Build history of the part. All positions in model axes, mm. Round coordinates to 2 decimals unless told otherwise and drop trailing zeros. Write each loop counter-clockwise with the first axis right and the second up, starting at its lowest first coordinate (ties: lowest second). Pieces come first, ordered by that corner, then holes.
Item 1: Wall check: probe 1 along Z at (x, y) = (29.5, -0.25); probe 2 along Z at (x, y) = (25.5, 5.75); probe 3 along Y at (x, z) = (-30, 10). Give the ranges that are in metal, low to high.
Item 2: Band-saw the part on A-A, the plane z = 0. Write the cut outline in (x, y).
Item 3: Band-saw the part on B-B, the plane z = 76.5. Write the cut outline in (x, y), then the cut area to 3 significant figures.
Item 4: Mould opens along Y. For faces 1 (the flat face through (0, -10, 1)), 2 (the cylindrical face through (23.979, 0.084, -46.757)), 3 (the flat face through (-29, -6, 1)) say: +Y half, -Y half, draft (parallel to the pull), parting line (faces both ways), or undercut.
Item 5: Drop flat-ended pins along their axis: pin 1 Ø2.5 at (y, z) = (0, -10) entering from +X; pin 2 Ø3 at (y, z) = (0, 10) entering from +X; pin 3 Ø2 at (y, z) = (0, 10) entering from +X. Give the stop position or say it passes through.
```python
from build123d import *

# Parameters (mm, degrees)
EXTRUDE_1_DEPTH             = 105
HOLE_WIZARD_M4_1_AT_2_COUNT = 2
HOLE_WIZARD_M4_1_AT_2_PITCH = 20
PATTERN_LINEAR_1_COUNT      = 3
PATTERN_LINEAR_1_PITCH      = 50
PATTERN_LINEAR_1_COUNT_DIR2 = 2
PATTERN_LINEAR_1_PITCH_DIR2 = 50


with BuildPart() as part:
    # 草图1 → 凸台-拉伸1 (new, symmetric)
    with BuildSketch(Plane.XY):
        Polygon((-25, -10), (25, -10), (15, -6), (37.5, -6), (37.5, 6), (-37.5, 6), (-37.5, -6), (-15, -6), align=None)
    extrude(amount=EXTRUDE_1_DEPTH, both=True)

    # 草图2 → M4 螺纹孔1 (revolve, cut)
    with BuildSketch(Plane(origin=(-37.5, 0, -10), x_dir=(0, 0, 1), z_dir=(0, 1, 0))):
        Polygon((0, 0), (0, 11.091420021), (1.65, 10.1), (1.65, 0), align=None)
    hole_wizard_m4_1 = revolve(axis=Axis((-43.85, 0, -10), (1, 0, 0)), mode=Mode.SUBTRACT)

    # M4 螺纹孔1 at 2: M4 螺纹孔1 ×2
    with Locations(*[(0, 0, i * HOLE_WIZARD_M4_1_AT_2_PITCH) for i in range(1, HOLE_WIZARD_M4_1_AT_2_COUNT)]):
        add(hole_wizard_m4_1, mode=Mode.SUBTRACT)

    # 镜向1: M4 螺纹孔1 across plane
    add(hole_wizard_m4_1.mirror(Plane(origin=(0, 0, 0), x_dir=(0, 0, 1), z_dir=(1, 0, 0))), mode=Mode.SUBTRACT)

    # 镜向1 copy 1 sketch → 镜向1 copy 1 (revolve, cut)
    with BuildSketch(Plane(origin=(37.5, 0, 10), x_dir=(0, 0, 1), z_dir=(0, 1, 0))):
        Polygon((0, 0), (0, -11.091420021), (1.65, -10.1), (1.65, 0), align=None)
    revolve(axis=Axis((43.85, 0, 10), (1, 0, 0)), mode=Mode.SUBTRACT)

    # 草图4 → M8 螺纹孔1 (revolve, cut)
    with BuildSketch(Plane(origin=(-25, 6, -50), x_dir=(0, 0, 1), z_dir=(1, 0, 0))):
        Polygon((0, 0), (0, 21.792926105), (3.4, 19.75), (3.4, 0), align=None)
    hole_wizard_m8_1 = revolve(axis=Axis((-25, 12.35, -50), (0, -1, 0)), mode=Mode.SUBTRACT)

    # 阵列(线性)1: Hole Wizard M8 _1 3 × 2
    with Locations(*[(j * PATTERN_LINEAR_1_PITCH_DIR2, 0, i * PATTERN_LINEAR_1_PITCH) for i in range(PATTERN_LINEAR_1_COUNT) for j in range(PATTERN_LINEAR_1_COUNT_DIR2) if (i, j) != (0, 0)]):
        add(hole_wizard_m8_1, mode=Mode.SUBTRACT)


solid = part.part
```
Results:
1. probe 1: z = -105 to -11.63, -8.37 to 8.37, 11.63 to 105
1. probe 2: z = -105 to -53.36, -46.64 to -3.36, 3.36 to 46.64, 53.36 to 105
1. probe 3: y = -6 to -1.65, 1.65 to 6
2. outline: (-37.5, -6) - (-28.4, -6) - (-28.4, 6) - (-37.5, 6) - close; (-21.6, -10) - (21.6, -10) - (21.6, -8.64) - (15, -6) - (21.6, -6) - (21.6, 6) - (-21.6, 6) - (-21.6, -6) - (-15, -6) - (-21.6, -8.64) - close; (28.4, -6) - (37.5, -6) - (37.5, 6) - (28.4, 6) - close
3. outline: (-37.5, -6) - (-15, -6) - (-25, -10) - (25, -10) - (15, -6) - (37.5, -6) - (37.5, 6) - (-37.5, 6) - close
3. area: 1,060 mm2
4. face 1: -Y half
4. face 2: draft
4. face 3: undercut
5. pin 1: stops at x = 27.16
5. pin 2: stops at x = 27.31
5. pin 3: stops at x = 27.01
